```python
from build123d import *

# Parameters (mm, degrees)
SKETCH1_R           = 27.5
SKETCH1_R_2         = 17.5
BOSS_EXTRUDE1_DEPTH = 100
SKETCH2_R           = 35.5
BOSS_EXTRUDE2_DEPTH = 21.35
SKETCH3_R           = 11
BOSS_EXTRUDE3_DEPTH = 85
SKETCH4_R           = 15
BOSS_EXTRUDE4_DEPTH = 165
SKETCH5_R           = 10
BOSS_EXTRUDE5_DEPTH = 15


with BuildPart() as part:
    # Sketch1 → Boss-Extrude1 (new body)
    with BuildSketch(Plane.XY):
        Circle(SKETCH1_R)
        Circle(SKETCH1_R_2, mode=Mode.SUBTRACT)
    extrude(amount=BOSS_EXTRUDE1_DEPTH)

    # Sketch2 → Boss-Extrude2 (add)
    with BuildSketch(Plane.XY.offset(100)):
        with Locations(Location((0, 0, 0), (0, 0, 180))):
            Circle(SKETCH2_R)
    extrude(amount=BOSS_EXTRUDE2_DEPTH)

    # Sketch3 → Boss-Extrude3 (add)
    with BuildSketch(Plane.XY.offset(121.35)):
        Circle(SKETCH3_R)
    extrude(amount=BOSS_EXTRUDE3_DEPTH)

    # Sketch4 → Boss-Extrude4 (add)
    with BuildSketch(Plane.XY.offset(206.35)):
        Circle(SKETCH4_R)
    extrude(amount=BOSS_EXTRUDE4_DEPTH)

    # Sketch5 → Boss-Extrude5 (add)
    with BuildSketch(Plane.XY.offset(371.35)):
        Circle(SKETCH5_R)
    extrude(amount=BOSS_EXTRUDE5_DEPTH)


solid = part.part
```
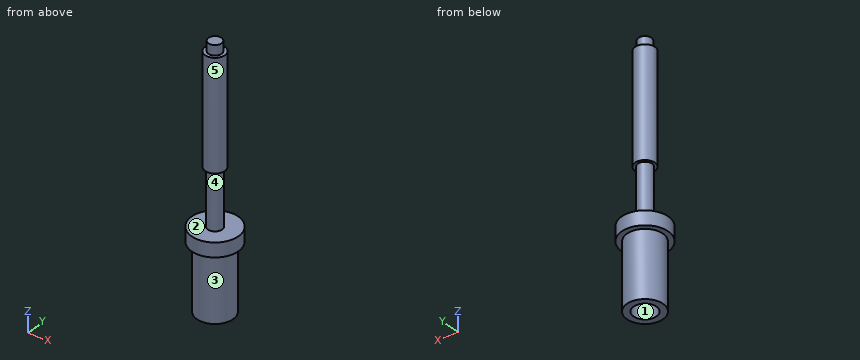
For this review, take the finished solid that the model builds, in its own axes (mm). Face numbers are marked on the shaded views. A direction names the side the tool comes from. Round coordinates to 2 decimals unless told otherwise and drop trailing zeros. Write each loop counter-clockwise with the first axis right and the second up, starting at its lowest first coordinate (ties: lowest second). Pieces come first, ordered by that corner, then holes. Notation, with made-up numbers: (-13, -18) - (-7, -18) arc R28 ccw to (-7, 3) - close; hole circle Ø4 at (76.5, 68). An arc over 180 degrees is marked (long way). Write each question's results on one line, items separated by ' | '.
Item 1: Draft analysis for pull direction Y (two halves, no side actions). For the marked faces 1, 2 and 3, state which applies: pulls with the +Y half, pulls with the -Y half, needs draft (parallel to the pull), parting line crosses it, or undercut.
Calculated:
face 1: undercut | face 2: needs draft | face 3: parting line crosses it
Item 2: Take a section at A-A on y = 0. State the section outline as (x, z) points.
Calculated:
outline: (-35.5, 100) - (-27.5, 100) - (-27.5, 0) - (-17.5, 0) - (-17.5, 100) - (17.5, 100) - (17.5, 0) - (27.5, 0) - (27.5, 100) - (35.5, 100) - (35.5, 121.35) - (11, 121.35) - (11, 206.35) - (15, 206.35) - (15, 371.35) - (10, 371.35) - (10, 386.35) - (-10, 386.35) - (-10, 371.35) - (-15, 371.35) - (-15, 206.35) - (-11, 206.35) - (-11, 121.35) - (-35.5, 121.35) - close
Item 3: Take a section at C-C on z = 348.5. State the section outline as (x, y) points, then the cut area to 3 significant figures.
Calculated:
outline: circle Ø30 at (0, 0) | area: 707 mm^2
Item 4: To check wall thickness, follow line 1 along Y through (x, z) = (0, 61); line 2 along Z through (x, y) = (10, -6); line 3 along Z through (x, y) = (-26.5, 18.5). State the ranges of each line that lie inside material, in increasing order. Write a range as from..to.
Calculated:
line 1: y = -27.5..-17.5, 17.5..27.5 | line 2: z = 100..121.35, 206.35..371.35 | line 3: z = 100..121.35
Item 5: For pin 1 (15 mm diameter, centred on x = 4, y = 7, fed in from -Z); pin 2 (5 mm diameter, centred on x = -10.5, y = 9.5, fed in from +Z); pin 3 (12 mm diameter, centred on x = 0, z = 124.5, fed in from +Y), all flat-tipped, find the tip position at first contact; note any pin that passes through.
Calculated:
pin 1: stops at z = 100 | pin 2: stops at z = 371.35 | pin 3: stops at y = 35.5
Item 6: For the marked faces 4 and 5, list the 3-axis set-ups (+Z, -Z, +X, -X, +Y, -Y) from which the entire face can be reached by the end or side of a thin tool; tool diameter is ignored.
Calculated:
face 4: none | face 5: +Z
